Could you check a few things on this model? Use its own coordinates, in mm. Coordinates: 2 decimals unless noted, no trailing zeros. Loops run counter-clockwise (first coordinate to the right, second up) from the corner with the lowest first, then second, coordinate; pieces in that order, holes last. Notation, with made-up numbers: (3.25, 23.25) - (36.25, 23.25) arc R8 ccw to (36.25, 27.25) - close; hole circle Ø6 at (-2, 77). An arc over 180 degrees is marked (long way). Use CSV: the item, a comma, the result in double quotes.
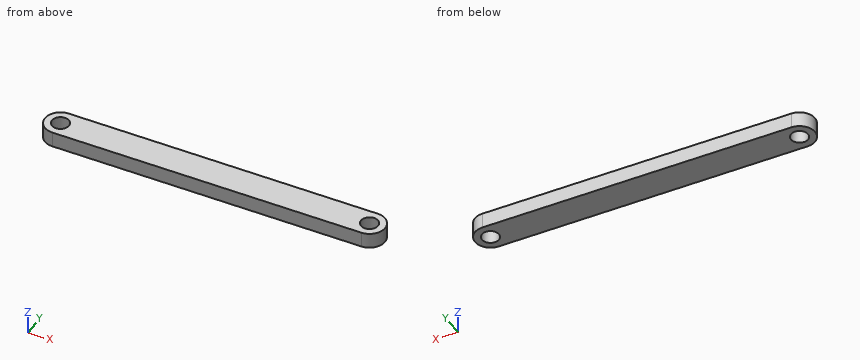
from build123d import *

# Parameters (mm, degrees)
SKETCH1_R           = 0.55
THIGH1_LENGTH_DEPTH = 0.5


with BuildPart() as part:
    # Sketch1 → Thigh1 length (new, symmetric)
    with BuildSketch(Plane.XY):
        with BuildLine():
            Line((-10, 1), (10, 1))
            ThreePointArc((10, 1), (11, 0), (10, -1))
            Line((10, -1), (-10, -1))
            ThreePointArc((-10, -1), (-11, 0), (-10, 1))
        make_face()
        with Locations((-10, 0)):
            Circle(SKETCH1_R, mode=Mode.SUBTRACT)
        with Locations((10, 0)):
            Circle(SKETCH1_R, mode=Mode.SUBTRACT)
    extrude(amount=THIGH1_LENGTH_DEPTH, both=True)


solid = part.part
(1) Suppose I cut it at A-A (z = -0.1). Write out the boundary of the cut face in (x, y).
Computed:
outline,"(-10, -1) - (10, -1) arc R1 ccw to (10, 1) - (-10, 1) arc R1 ccw to start; hole circle Ø1.1 at (-10, 0); hole circle Ø1.1 at (10, 0)"
(2) Suppose I cut it at B-B (y = -0.3). Write out the boundary of the cut face in (x, z), plus the area to 3 significant figures.
Computed:
outline,"(-10.95, -0.5) - (-10.46, -0.5) - (-10.46, 0.5) - (-10.95, 0.5) - close; (-9.54, -0.5) - (9.54, -0.5) - (9.54, 0.5) - (-9.54, 0.5) - close; (10.46, -0.5) - (10.95, -0.5) - (10.95, 0.5) - (10.46, 0.5) - close"
area,"20.1 mm²"
(3) Please list where these lines run through material, in increasing order: line 1 (Y direction, x = -10, z = 0.35); line 2 (X direction, y = 0.4, z = 0); line 3 (X direction, y = 0.1, z = -0.15).
Computed:
line 1,"y = -1 to -0.55, 0.55 to 1"
line 2,"x = -10.92 to -10.38, -9.62 to 9.62, 10.38 to 10.92"
line 3,"x = -10.99 to -10.54, -9.46 to 9.46, 10.54 to 10.99"
